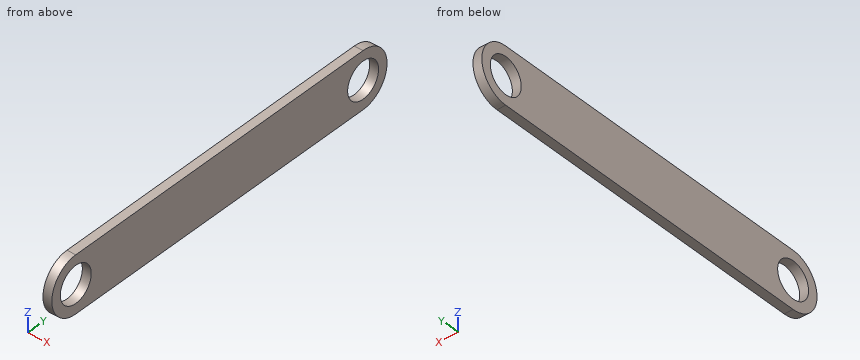
```python
from build123d import *

# Parameters (mm, degrees)
SKETCH1_R           = 4.1
BOSS_EXTRUDE1_DEPTH = 2


with BuildPart() as part:
    # Sketch1 → Boss-Extrude1 (new body)
    with BuildSketch(Plane(origin=(0, 0, 0), x_dir=(0, 0, -1), z_dir=(1, 0, 0))):
        with BuildLine():
            Line((-6.35, -38.1), (-6.35, 38.1))
            ThreePointArc((-6.35, 38.1), (0, 44.45), (6.35, 38.1))
            Line((6.35, 38.1), (6.35, -38.1))
            ThreePointArc((6.35, -38.1), (0, -44.45), (-6.35, -38.1))
        make_face()
        with Locations((0, 38.1)):
            Circle(SKETCH1_R, mode=Mode.SUBTRACT)
        with Locations((0, -38.1)):
            Circle(SKETCH1_R, mode=Mode.SUBTRACT)
    extrude(amount=BOSS_EXTRUDE1_DEPTH)


solid = part.part
```
Model file for the job. Use its own axes, mm. Coordinates: 2 decimals unless noted, no trailing zeros. Loops run counter-clockwise (first coordinate to the right, second up) from the corner with the lowest first, then second, coordinate; pieces in that order, holes last. Notation, with made-up numbers: (-30, -1) - (6, -1) arc R25 cw to (6, 27) - close; hole circle Ø8 at (43.25, 5). An arc over 180 degrees is marked (long way). Write item = value, one per line. Start each with the question number.
Item 1: Saw through at C-C, the plane x = 0.9. List the corners of the cut face in (y, z).
Item 2: Wall check: probe 1 along Y at (x, z) = (0.5, 0); probe 2 along Y at (x, z) = (1.6, 1.25); probe 3 along Z at (x, y) = (1.7, 35.5). Give the ranges that are in metal, low to high. Write a range as [from, to].
Item 3: Saw through at D-D, the plane z = 5.5. List the corners of the cut face in (x, y).
Item 4: Drop a flat-ended pin along its axis: pin 1 Ø1 at (x, z) = (0, -2) entering from +Y. Give the stop position or say it passes through.
Item 5: Saw through at B-B, the plane y = -36.5. List the corners of the cut face in (x, z), then the cut area to 3 significant figures.
Item 6: Saw through at A-A, the plane z = 0. List the corners of the cut face in (x, y), then the cut area to 3 significant figures.
Answers:
q1.outline = (-38.1, -6.35) - (38.1, -6.35) arc R6.35 ccw to (38.1, 6.35) - (-38.1, 6.35) arc R6.35 ccw to start; hole circle Ø8.2 at (-38.1, 0); hole circle Ø8.2 at (38.1, 0)
q2.probe_1 = [-44.45, -42.2], [-34, 34], [42.2, 44.45]
q2.probe_2 = [-44.33, -42], [-34.2, 34.2], [42, 44.33]
q2.probe_3 = [-6.35, -3.17], [3.17, 6.35]
q3.outline = (0, -41.27) - (2, -41.27) - (2, 41.27) - (0, 41.27) - close
q4.pin_1 = 44.27
q5.outline = (0, -6.35) - (2, -6.35) - (2, -3.77) - (0, -3.77) - close; (0, 3.77) - (2, 3.77) - (2, 6.35) - (0, 6.35) - close
q5.area = 10.3 mm2
q6.outline = (0, -44.45) - (2, -44.45) - (2, -42.2) - (0, -42.2) - close; (0, -34) - (2, -34) - (2, 34) - (0, 34) - close; (0, 42.2) - (2, 42.2) - (2, 44.45) - (0, 44.45) - close
q6.area = 145 mm2
